from build123d import *

# Parameters (mm, degrees)
EXTRUDE_1_DEPTH     = 10
SKETCH_2_R          = 6.25
CUT_EXTRUDE_1_DEPTH = 220.431082575
CHAMFER_1_SIZE      = 2


with BuildPart() as part:
    # 草图1 → 凸台-拉伸1 (new body)
    with BuildSketch(Plane.XY):
        with BuildLine():
            Line((-82.5, 100.5), (82.5, 100.5))
            ThreePointArc((82.5, 100.5), (95.227922061, 95.227922061), (100.5, 82.5))
            Line((100.5, 82.5), (100.5, 2.5))
            Line((100.5, 2.5), (155, 2.5))
            Line((155, 2.5), (155, 135))
            ThreePointArc((155, 135), (149.142135624, 149.142135624), (135, 155))
            Line((135, 155), (-135, 155))
            ThreePointArc((-135, 155), (-149.142135624, 149.142135624), (-155, 135))
            Line((-155, 135), (-155, 2.5))
            Line((-155, 2.5), (-100.5, 2.5))
            Line((-100.5, 2.5), (-100.5, 82.5))
            ThreePointArc((-100.5, 82.5), (-95.227922061, 95.227922061), (-82.5, 100.5))
        make_face()
    extrude(amount=EXTRUDE_1_DEPTH)

    # 草图2 → 切除-拉伸1 (cut, through all)
    with BuildSketch(Plane.XY.offset(10)):
        with Locations((0, 137)):
            Circle(SKETCH_2_R)
        with Locations((0, -137)):
            Circle(SKETCH_2_R)
        with Locations((-137, 137)):
            Circle(SKETCH_2_R)
        with Locations((137, 137)):
            Circle(SKETCH_2_R)
        with Locations((-137, -137)):
            Circle(SKETCH_2_R)
        with Locations((137, -137)):
            Circle(SKETCH_2_R)
        with Locations((-137, 15)):
            Circle(SKETCH_2_R)
        with Locations((-137, -15)):
            Circle(SKETCH_2_R)
        with Locations((137, -15)):
            Circle(SKETCH_2_R)
        with Locations(Location((137, 15, 0), (0, 0, 180))):
            Circle(SKETCH_2_R)
    extrude(amount=-CUT_EXTRUDE_1_DEPTH, mode=Mode.SUBTRACT)

    # 倒角1
    chamfer_1_edges = [part.edges().sort_by_distance(p)[0] for p in [
        (-100.5, 2.5, 5),
        (-155, 2.5, 5),
        (155, 2.5, 5),
        (100.5, 2.5, 5),
    ]]
    chamfer(chamfer_1_edges, length=CHAMFER_1_SIZE)


solid = part.part
Could you check a few things on this model? Use its own coordinates, in mm. A direction names the side the tool comes from. Give positions to 0.01 mm unless a question says otherwise; leave off trailing zeros. Order: outer loops, then holes, each group sorted by start corner. A loop starts at its lowest first (then second) coordinate and runs counter-clockwise, first axis right, second up. Notation, with made-up numbers: (65.25, -29) - (104.25, -29) arc R34 ccw to (104.25, 4) - close; hole circle Ø7 at (31, 16). An arc over 180 degrees is marked (long way). Return JSON: item names as keys, results as strings. Group by question number.
Q1. Thinking about a two-plate mould opening in X: for faces 3 (the face through (-95.367, 95.087, 4.93)), 4 (the face through (-128, 2.5, 5)), 5 (the face through (149.297, 148.986, 4.93)), 6 (the face through (-148.986, 149.297, 4.93)), which applies, pulls with the +X half, pulls with the -X half, needs draft (parallel to the pull), parting line crosses it, or undercut?
Q2. Will these pins go through, and if not, where does the flat tip stop? pin 1 Ø7.5 at (x, y) = (0, 137) entering from -Z; pin 2 Ø5 at (x, z) = (26, 4) entering from -Y.
Q3. Suppose I cut it at A-A, the plane y = 38. Please give me the cut outline in (x, z).
Q4. Please list where these lines run through material, in increasing order: line 1 along Y through (x, z) = (-137, 8.25); line 2 along X through (y, z) = (68.5, 4.5); line 3 along X through (y, z) = (131.5, 9.5). Write a range as [from, to].
Q5. Which directions (+Z, -Z, +X, -X, +Y, -Y) give clear straight access to the entire face, cutting with the end or side of a thin tool? Please do faces 1 (the face through (100.5, 44, 5)), 2 (the face through (-2, 114, 0)).
Q6. Suppose I cut it at B-B, the plane x = 0. Please give me the cut outline in (y, z).
Q7. Suppose I cut it at C-C, the plane z = 2.75. Please give me the cut outline in (x, y), and give its area (3 significant figures).
Q8. Suppose I cut it at D-D, the plane x = -39.5. Please give me the cut outline in (y, z), and give its area (3 significant figures).
Resolved:
{
 "1": {"face 3": "undercut", "face 4": "needs draft", "face 5": "pulls with the +X half", "face 6": "pulls with the -X half"},
 "2": {"pin 1": "passes through", "pin 2": "stops at y = 100.5"},
 "3": {"outline": "(-155, 0) - (-100.5, 0) - (-100.5, 10) - (-155, 10) - close; (100.5, 0) - (155, 0) - (155, 10) - (100.5, 10) - close"},
 "4": {"line 1": "y = [2.5, 8.75], [21.25, 130.75], [143.25, 154.9]", "line 2": "x = [-155, -100.5], [100.5, 155]", "line 3": "x = [-155, -139.97], [-134.03, -2.97], [2.97, 134.03], [139.97, 155]"},
 "5": {"face 1": "+Z, -Z, -Y", "face 2": "-Z, +X, -X, +Y, -Y"},
 "6": {"outline": "(100.5, 0) - (130.75, 0) - (130.75, 10) - (100.5, 10) - close; (143.25, 0) - (155, 0) - (155, 10) - (143.25, 10) - close"},
 "7": {"outline": "(-155, 4.5) - (-153, 2.5) - (-102.5, 2.5) - (-100.5, 4.5) - (-100.5, 82.5) arc R18 cw to (-82.5, 100.5) - (82.5, 100.5) arc R18 cw to (100.5, 82.5) - (100.5, 4.5) - (102.5, 2.5) - (153, 2.5) - (155, 4.5) - (155, 135) arc R20 ccw to (135, 155) - (-135, 155) arc R20 ccw to (-155, 135) - close; hole circle Ø12.5 at (-137, 15); hole circle Ø12.5 at (-137, 137); hole circle Ø12.5 at (0, 137); hole circle Ø12.5 at (137, 15); hole circle Ø12.5 at (137, 137)", "area": "26,900 mm2"},
 "8": {"outline": "(100.5, 0) - (155, 0) - (155, 10) - (100.5, 10) - close", "area": "545 mm2"}
}
